Check sheet for the modelled part. Datum: model origin and axes. Units: mm. Give positions to 0.01 mm unless a question says otherwise; leave off trailing zeros. Order: outer loops, then holes, each group sorted by start corner. A loop starts at its lowest first (then second) coordinate and runs counter-clockwise, first axis right, second up. Notation, with made-up numbers: M 31,8.5 L 80,8.5 A27 ccw 80,25.5 Z; hole C -6.5,-11.75 d5. An arc over 180 degrees is marked long. Answer in a Markdown table with one row per item. Add a question column.
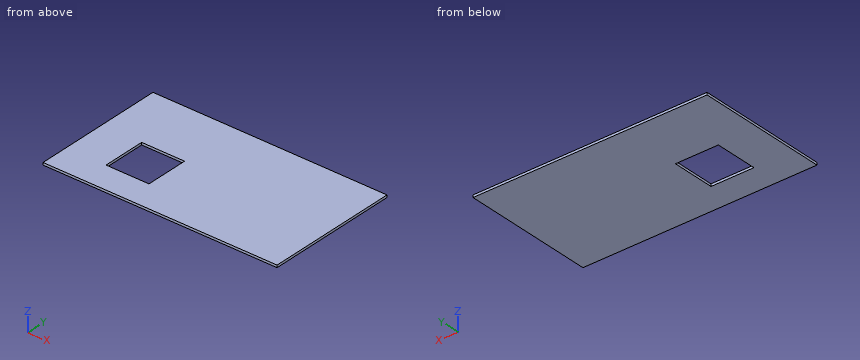
from build123d import *

# Parameters (mm, degrees)
SKETCH1_W           = 300
SKETCH1_H           = 170
BOSS_EXTRUDE1_DEPTH = 3
SKETCH2_W           = 55
SKETCH2_H           = 55
CUT_EXTRUDE2_DEPTH  = 40.5


with BuildPart() as part:
    # Sketch1 → Boss-Extrude1 (new body)
    with BuildSketch(Plane.XY):
        with Locations((-20, 0)):
            Rectangle(SKETCH1_W, SKETCH1_H)
    extrude(amount=BOSS_EXTRUDE1_DEPTH)

    # Sketch2 → Cut-Extrude2 (cut)
    with BuildSketch(Plane(origin=(0, 0, 0), x_dir=(-1, 0, 0), z_dir=(0, 0, -1))):
        with Locations((91.5, -21.5)):
            Rectangle(SKETCH2_W, SKETCH2_H)
    extrude(amount=-CUT_EXTRUDE2_DEPTH, mode=Mode.SUBTRACT)


solid = part.part
Q1. Cross-section at A-A (y = -10). Record the boundary of the cut face in (x, z).
Q2. Cross-section at B-B (z = 1.2). Record the boundary of the cut face in (x, y), and give its area (3 significant figures).
Q3. Thickness scan on probe 1 along Y at (x, z) = (-87, 0.5); probe 2 along X at (y, z) = (-40.5, 2.4). Record the ranges inside material, lowest first.
Q4. Cross-section at C-C (x = -109). Record the boundary of the cut face in (y, z).
Values follow:
| question | item | result |
|---|---|---|
| 1 | outline | M -170,0 L -119,0 L -119,3 L -170,3 Z; M -64,0 L 130,0 L 130,3 L -64,3 Z |
| 2 | outline | M -170,-85 L 130,-85 L 130,85 L -170,85 Z; hole M -119,-49 L -64,-49 L -64,6 L -119,6 Z |
| 2 | area | 48,000 mm² |
| 3 | probe 1 | -85 to -49, 6 to 85 |
| 3 | probe 2 | -170 to -119, -64 to 130 |
| 4 | outline | M -85,0 L -49,0 L -49,3 L -85,3 Z; M 6,0 L 85,0 L 85,3 L 6,3 Z |
